The drawing under review shows one solid part. Ordinate dimensions are in mm from its lowest x, y, z. A direction names the side the tool comes from. Coordinates: 2 decimals unless noted, no trailing zeros. Write each loop counter-clockwise with the first axis right and the second up, starting at its lowest first coordinate (ties: lowest second). Pieces come first, ordered by that corner, then holes.
Q1. Clearance check with flat-ended pins moving along their axes: pin 1 Ø8 at (x, y) = (31.61, 17.83) entering from +Z; pin 2 Ø3.5 at (x, y) = (18, 14.5) entering from +Z. State where each tip first meets the part, or that it passes through.
Q2. Add section B-B, the plane y = 47. Give the boundary of the cut face in (x, z), plus the area to 3 significant figures.
Q3. Add section A-A, the plane z = 6.5. Give the boundary of the cut face in (x, y), plus the area to 3 significant figures.
Q4. The part is to be moulded in two halves that separate along Y. For the marked faces 3, 4 and 5, say which applies: +Y half, -Y half, draft (parallel to the pull), parting line (faces both ways), or undercut.
Q5. Add section C-C, the plane x = 18.5. Give the number of separate pieces and of enclosed holes in the cut face, plus the area to 3 significant figures.
Q6. To check wall thickness, follow probe 1 along Y at (x, z) = (19, 2.5); probe 2 along Y at (x, z) = (16.5, 5.75); probe 3 along Y at (x, z) = (16.5, 16). State the ranges of each line that lie inside material, in increasing order.
Q7. Machinability: for the marked faces 1 and 2, which of the approach directions +Z, -Z, +X, -X, +Y, -Y give a long, thin tool a straight path to every point of the face, cutting with its end or side? Answer none if there is none.
Q8. Add section D-D, the plane y = 14. Give the boundary of the cut face in (x, z), plus the area to 3 significant figures.
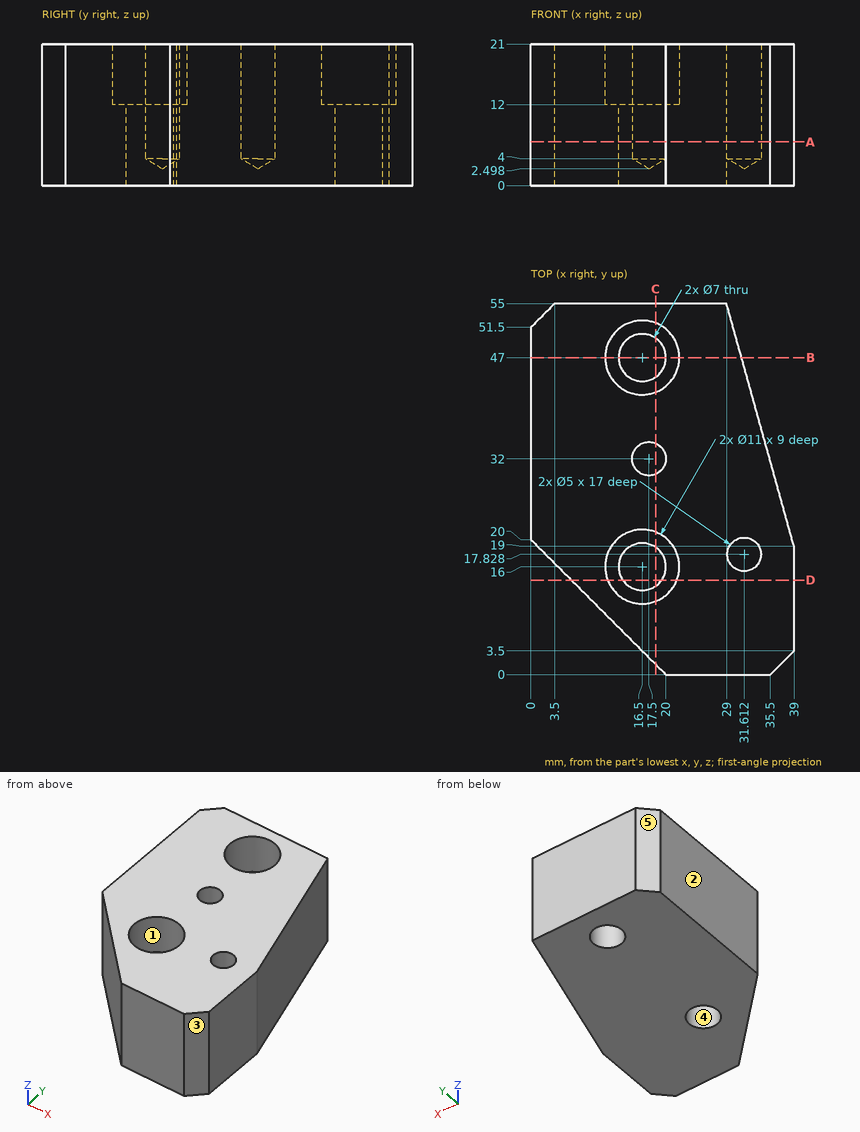
Here are the results:
1. pin 1: stops at z = 21
1. pin 2: stops at z = 12
2. outline: (0, 0) - (13, 0) - (13, 12) - (11, 12) - (11, 21) - (0, 21) - close; (20, 0) - (31.22, 0) - (31.22, 21) - (22, 21) - (22, 12) - (20, 12) - close
2. area: 473 mm2
3. outline: (0, 20) - (20, 0) - (35.5, 0) - (39, 3.5) - (39, 19) - (29, 55) - (3.5, 55) - (0, 51.5) - close; hole circle Ø7 at (16.5, 16); hole circle Ø7 at (16.5, 47); hole circle Ø5 at (17.5, 32); hole circle Ø5 at (31.61, 17.83)
3. area: 1,640 mm2
4. face 3: -Y half
4. face 4: undercut
4. face 5: +Y half
5. separate pieces: 3
5. enclosed holes: 0
5. area: 721 mm2
6. probe 1: y = 1 to 13.55, 18.45 to 44.55, 49.45 to 55
6. probe 2: y = 3.5 to 12.5, 19.5 to 29.71, 34.29 to 43.5, 50.5 to 55
6. probe 3: y = 3.5 to 10.5, 21.5 to 29.71, 34.29 to 41.5, 52.5 to 55
7. face 1: +Z
7. face 2: +Z, -Z, -X, +Y, -Y
8. outline: (6, 0) - (13.63, 0) - (13.63, 12) - (11.38, 12) - (11.38, 21) - (6, 21) - close; (19.37, 0) - (39, 0) - (39, 21) - (21.62, 21) - (21.62, 12) - (19.37, 12) - close
8. area: 532 mm2
